Study the drawing (mm; zero at the part's minimum x, y, z) and answer. Round coordinates to 2 decimals unless told otherwise and drop trailing zeros. Write each loop counter-clockwise with the first axis right and the second up, starting at its lowest first coordinate (ties: lowest second). Pieces come first, ordered by that corner, then holes. Notation, with made-up numbers: (1.5, -11.5) - (38.5, -11.5) arc R5 ccw to (38.5, -6.5) - close; hole circle Ø10 at (-14.75, 44). An arc over 180 degrees is marked (long way). Return JSON: item names as keys, results as strings. Group by question number.
(1) Each of these flat-tipped pins is pushed along its axis until it touches: pin 1 (8 mm diameter, centred on y = 3.5, z = 49.5, fed in from -X); pin 2 (5.5 mm diameter, centred on y = 10, z = 36, fed in from +X). Where does it stop, or does it pass through?
(2) Determine the mould class of the marked faces 1, 2, 3 and 4 for opening direction Z: +Z half, -Z half, draft (parallel to the pull), parting line (faces both ways), or undercut.
(3) Find the intervals of material crossed by line 1 along Z through (x, y) = (4, 9.75); line 2 along Y through (x, z) = (5.5, 84); line 3 along Z through (x, y) = (8.25, 13.5), in increasing order. Write a range as [from, to].
(4) Section D-D, the plane y = 15.5 is taken. Write down the section's boundary in (x, z).
(5) Section B-B, the plane x = 8.25 is taken. Write down the section's boundary in (y, z).
(6) Section A-A, the plane y = 10 is taken. Write down the section's boundary in (x, z).
(7) Section C-C, the plane z = 110 is taken. Write down the section's boundary in (x, y), then the cut area to 3 significant figures.
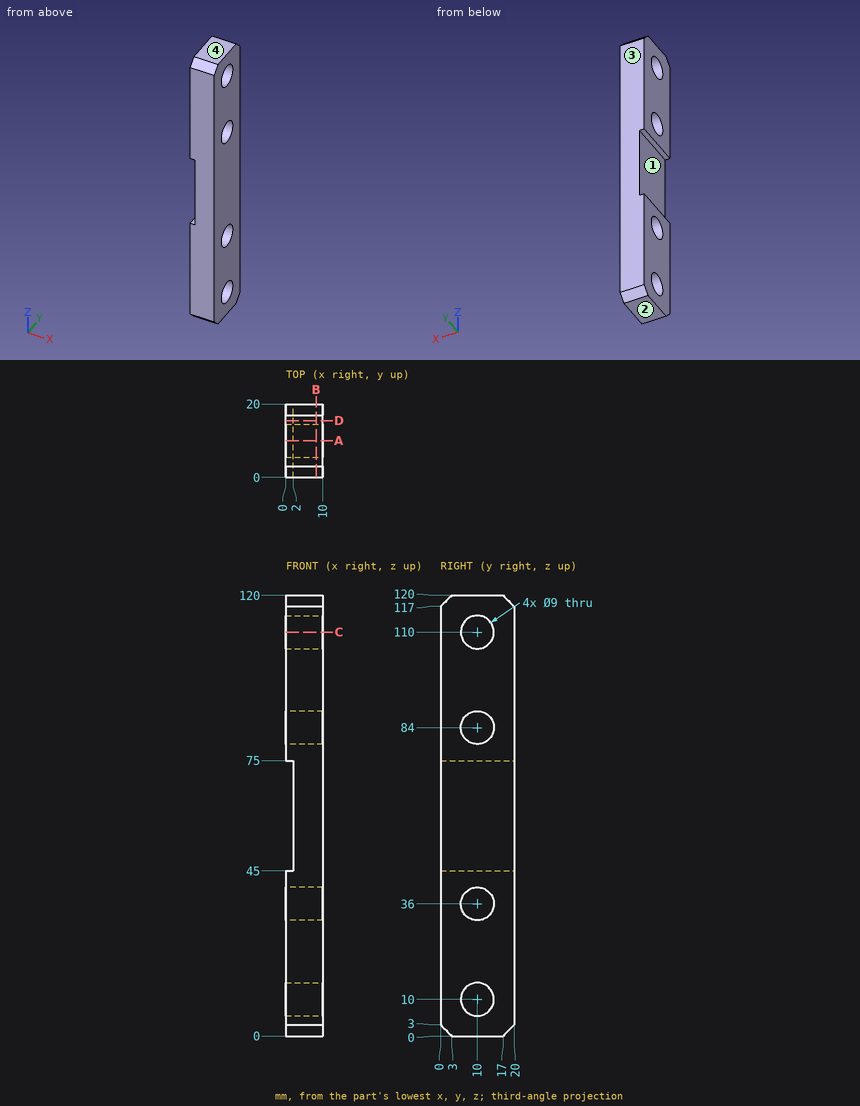
Working result:
{
 "1": {"pin 1": "stops at x = 2", "pin 2": "passes through"},
 "2": {"face 1": "undercut", "face 2": "-Z half", "face 3": "draft", "face 4": "+Z half"},
 "3": {"line 1": "z = [0, 5.51], [14.49, 31.51], [40.49, 79.51], [88.49, 105.51], [114.49, 120]", "line 2": "y = [0, 5.5], [14.5, 20]", "line 3": "z = [0, 7.17], [12.83, 33.17], [38.83, 81.17], [86.83, 107.17], [112.83, 120]"},
 "4": {"outline": "(0, 0) - (10, 0) - (10, 120) - (0, 120) - (0, 75) - (2, 75) - (2, 45) - (0, 45) - close"},
 "5": {"outline": "(0, 3) - (3, 0) - (17, 0) - (20, 3) - (20, 117) - (17, 120) - (3, 120) - (0, 117) - close; hole circle Ø9 at (10, 10); hole circle Ø9 at (10, 36); hole circle Ø9 at (10, 84); hole circle Ø9 at (10, 110)"},
 "6": {"outline": "(0, 0) - (10, 0) - (10, 5.5) - (0, 5.5) - close; (0, 14.5) - (10, 14.5) - (10, 31.5) - (0, 31.5) - close; (0, 40.5) - (10, 40.5) - (10, 79.5) - (0, 79.5) - (0, 75) - (2, 75) - (2, 45) - (0, 45) - close; (0, 88.5) - (10, 88.5) - (10, 105.5) - (0, 105.5) - close; (0, 114.5) - (10, 114.5) - (10, 120) - (0, 120) - close"},
 "7": {"outline": "(0, 0) - (10, 0) - (10, 5.5) - (0, 5.5) - close; (0, 14.5) - (10, 14.5) - (10, 20) - (0, 20) - close", "area": "110 mm^2"}
}
